For this review, take the finished solid that the model builds, in its own axes (mm). A direction names the side the tool comes from. Coordinates: 2 decimals unless noted, no trailing zeros. Loops run counter-clockwise (first coordinate to the right, second up) from the corner with the lowest first, then second, coordinate; pieces in that order, holes last. Notation, with made-up numbers: M 41.25,27 L 73.25,27 A30 ccw 73.25,57 Z; hole C -17,7.5 d11. An arc over 180 degrees is marked long. Use one line per item in the form item = value.
```python
from build123d import *

# Parameters (mm, degrees)
SKETCH2_R          = 1.75
CUT_EXTRUDE1_DEPTH = 3
CHAMFER1_SIZE      = 1.5
CHAMFER2_SIZE      = 0.3


with BuildPart() as part:
    # Sketch1 → Revolve1 (revolve)
    with BuildSketch(Plane.XY, mode=Mode.PRIVATE) as revolve1_sk:
        Polygon((0, 11), (0, 24), (3, 24), (3, 15), (5.5, 15), (5.5, 12.8), (1, 12.8), (1, 11), align=None)
    revolve(revolve1_sk.sketch.rotate(Axis((0, 0, 0), (1, 0, 0)), 90), axis=Axis((0, 0, 0), (1, 0, 0)))

    # Sketch2 → Cut-Extrude1 (cut)
    with BuildSketch(Plane(origin=(3, 0, 0), x_dir=(0, 0, -1), z_dir=(1, 0, 0))):
        with Locations((0, 19.5)):
            Circle(SKETCH2_R)
        with Locations((19.5, 0)):
            Circle(SKETCH2_R)
        with Locations((0, -19.5)):
            Circle(SKETCH2_R)
        with Locations((-19.5, 0)):
            Circle(SKETCH2_R)
    extrude(amount=-CUT_EXTRUDE1_DEPTH, mode=Mode.SUBTRACT)

    # Chamfer1
    chamfer1_edges = [part.edges().sort_by_distance(p)[0] for p in [
        (0, 19.5, 1.75),
        (0, 0, -17.75),
        (0, -19.5, 1.75),
        (0, 0, 21.25),
    ]]
    chamfer(chamfer1_edges, length=CHAMFER1_SIZE)

    # Chamfer2
    chamfer2_edges = [part.edges().sort_by_distance(p)[0] for p in [
        (3, 0, -24),
        (0, 0, -24),
        (0, 0, -11),
        (5.5, 0, -12.8),
        (5.5, 0, -15),
    ]]
    chamfer(chamfer2_edges, length=CHAMFER2_SIZE)


solid = part.part
```
1. Wall thickness on line 1 along Y through (x, z) = (2.4, 0); line 2 along Y through (x, z) = (0.5, 0); line 3 along Y through (x, z) = (3.55, 0): over which ranges is each line inside the solid? List them lowest first. Write a range as from..to.
Computed values:
line_1 = -24..-21.25, -17.75..-12.8, 12.8..17.75, 21.25..24
line_2 = -24..-22.25, -16.75..-11, 11..16.75, 22.25..24
line_3 = -15..-12.8, 12.8..15
2. Draft analysis for pull direction Z (two halves, no side actions). For faces 1 (the face through (1, -10, 6)), 2 (the face through (2.26, -17.765, 0.228)), 3 (the face through (3, -11, -11)), 4 (the face through (1.52, -7.21, 22.89)), state which applies: +Z half, -Z half, draft (parallel to the pull), parting line (faces both ways), or undercut.
Computed values:
face_1 = undercut
face_2 = undercut
face_3 = draft
face_4 = parting line
3. For pin 1 Ø1 at (y, z) = (-1, -18) entering from +X; pin 2 Ø6 at (y, z) = (12.5, 2.5) entering from +X; pin 3 Ø4.5 at (y, z) = (0, -19.5) entering from -X, all flat-tipped, find the tip position at first contact; note any pin that passes through.
Computed values:
pin_1 = 3
pin_2 = 5.5
pin_3 = 1
4. Tool access review of faces 5 (the face through (3.07, -3.84, 12.21)), 6 (the face through (2.26, 21.235, 0.228)): name each direction out of +Z, -Z, +X, -X, +Y, -Y from which nothing blocks a thin tool from reaching the whole face with its end or side.
Computed values:
face_5 = +X
face_6 = +X, -X
5. Consider section A-A on y = 0. State how many separate pieces and enclosed holes the cut face has, plus the area to 4 significant figures.
Computed values:
separate_pieces = 4
enclosed_holes = 0
area = 55.85 mm2
6. Consider section B-B on x = 3.6. Write out the cut boundary in (y, z), plus the area to 3 significant figures.
Computed values:
outline = C 0,0 d30; hole C 0,0 d25.6
area = 192 mm2
